```python
from build123d import *

# Parameters (mm, degrees)
EXTRUDE_368_DEPTH = 5.3
SKETCH_4_W        = 0.6
SKETCH_4_H        = 11.005553499
CHAMFER_1891_SIZE = 1
FILLET_1936_R     = 0.4


with BuildPart() as part:
    # 草图1 → Extrude 368 (new body)
    with BuildSketch(Plane(origin=(0, 0, 0), x_dir=(0, 0, -1), z_dir=(1, 0, 0))):
        Polygon((6.5, 3.75277675), (6.5, -3.75277675), (0, -7.505553499), (-6.5, -3.75277675), (-6.5, 3.75277675), (0, 7.505553499), align=None)
    extrude(amount=EXTRUDE_368_DEPTH)

    # 草图2 → 凸台-旋转1 (revolve)
    with BuildSketch(Plane.XY, mode=Mode.PRIVATE) as revolve_1_sk:
        Polygon((0, 0), (35.3, 0), (35.3, 2.9175), (35.3, 4), (0, 4), align=None)
    revolve(revolve_1_sk.sketch.rotate(Axis((0, 0, 0), (1, 0, 0)), 90), axis=Axis((0, 0, 0), (1, 0, 0)))

    # 草图3 → 切除-旋转1 (revolve, cut)
    with BuildSketch(Plane.XY):
        Polygon((0, 6.5), (3.46730793, 12.505553499), (3.46730793, 17.505553499), (-10, 17.505553499), (-10, 6.5), align=None)
    revolve(axis=Axis((0, 0, 0), (1, 0, 0)), mode=Mode.SUBTRACT)

    # 草图5 → 切除-旋转2 (revolve, cut)
    with BuildSketch(Plane.XY):
        Polygon((5.3, 6.5), (1.83269207, 12.505553499), (1.83269207, 17.505553499), (11.83269207, 17.505553499), (11.83269207, 6.5), align=None)
    revolve(axis=Axis((0, 0, 0), (1, 0, 0)), mode=Mode.SUBTRACT)

    # 草图4 → 切除-旋转3 (revolve, cut)
    with BuildSketch(Plane.XY, mode=Mode.PRIVATE) as cut_revolve_3_sk:
        with Locations((5, 12.00277675)):
            Rectangle(SKETCH_4_W, SKETCH_4_H)
    revolve(cut_revolve_3_sk.sketch.rotate(Axis((0, 0, 0), (1, 0, 0)), 270), axis=Axis((0, 0, 0), (1, 0, 0)), mode=Mode.SUBTRACT)

    # Chamfer 1891
    chamfer_1891_edges = [part.edges().sort_by_distance(p)[0] for p in [
        (35.3, 0, -4),
    ]]
    chamfer(chamfer_1891_edges, length=CHAMFER_1891_SIZE)

    # Fillet 1936
    fillet_1936_edges = [part.edges().sort_by_distance(p)[0] for p in [
        (5.3, 0, -4),
    ]]
    fillet(fillet_1936_edges, radius=FILLET_1936_R)


solid = part.part
```
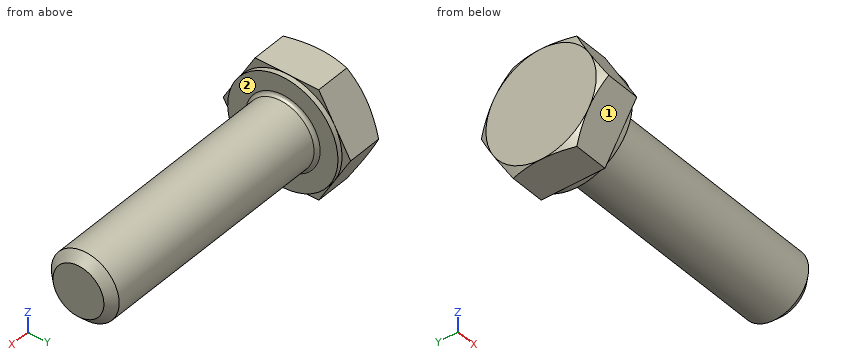
The model under review builds one solid part; all positions refer to its coordinate system, in mm. Face numbers are marked on the shaded views. A direction names the side the tool comes from. Round coordinates to 2 decimals unless told otherwise and drop trailing zeros. Loops run counter-clockwise (first coordinate to the right, second up) from the corner with the lowest first, then second, coordinate; pieces in that order, holes last. Notation, with made-up numbers: (37, 68.25) -> (74, 68.25) arc R15 ccw to (74, 82.25) -> close; hole circle Ø6 at (69, -35). An arc over 180 degrees is marked (long way). Answer as a JSON object with one key per item and string values. Group by question number.
1) For the marked faces 1 and 2, list the 3-axis set-ups (+Z, -Z, +X, -X, +Y, -Y) from which the entire face can be reached by the end or side of a thin tool; tool diameter is ignored.
2) We need section B-B on x = 11.5. Write out the cut boundary in (y, z).
3) We need section A-A on x = 4. Write out the cut boundary in (y, z).
4) For line 1 (X direction, y = -3.5, z = 5.25); line 2 (Y direction, x = 23, z = 0.25); line 3 (Z direction, x = 19, y = 3.25), list the stretches that pass through material, from the lowest coordinate up. Write a range as [from, to].
5) For pin 1 Ø3 at (x, z) = (5, -5) entering from +Y; pin 2 Ø4 at (y, z) = (4, -4) entering from -X; pin 3 Ø1.6 at (y, z) = (3.5, -5) entering from +X; pin 4 Ø3 at (x, z) = (7, -2) entering from -Y, all flat-tipped, find the tip position at first contact; note any pin that passes through.
Result set:
{
 "1": {"face 1": "-Z, +X, -X, -Y", "face 2": "+X"},
 "2": {"outline": "circle Ø8 at (0, 0)"},
 "3": {"outline": "(-7.51, 0) -> (-3.75, -6.5) -> (3.75, -6.5) -> (7.51, 0) -> (3.75, 6.5) -> (-3.75, 6.5) -> close"},
 "4": {"line 1": "[0, 5.3]", "line 2": "[-3.99, 3.99]", "line 3": "[-2.33, 2.33]"},
 "5": {"pin 1": "y = 5.48", "pin 2": "x = 0", "pin 3": "x = 5.3", "pin 4": "y = -3.97"}
}
